The listing builds one solid part. Answer for the finished solid, in the listing's coordinates (mm). Face numbers are marked on the shaded views. A direction names the side the tool comes from. Coordinates: 2 decimals unless noted, no trailing zeros. Loops run counter-clockwise (first coordinate to the right, second up) from the corner with the lowest first, then second, coordinate; pieces in that order, holes last. Notation, with made-up numbers: M -37.75,-37 L -27.75,-37 A24 cw -27.75,-9 Z; hole C -15,-24.75 d8. An arc over 180 degrees is marked long. Answer as a JSON object with one key per item and string values. Group by question number.
1. Straight lines are drawn through the part: L1, parallel to Z at x = 91, y = 9; L2, parallel to X at y = 14.5, z = 6; L3, parallel to Y at x = 291.5, z = -6. For each, find the intervals that lie inside material, in ascending order.
2. A cutting plane is placed at B-B on x = 130.5. Give the vertices of the cut face in (y, z).
3. For the marked faces 1, 2 and 3, determine the directions among +Z, -Z, +X, -X, +Y, -Y from which every point of the face is accessible in a straight line to the end or side of a thin tool.
4. Given pin 1 (1.3 mm diameter, centred on x = -60.5, y = 15.5, fed in from +Z); pin 2 (3 mm diameter, centred on x = -117, z = -2.5, fed in from +Y); pin 3 (3 mm diameter, centred on x = -58.5, z = -2, fed in from +Y); pin 4 (6 mm diameter, centred on y = 0.5, z = 4.5, fed in from +X), each flat-ended and moving along its own axis, determine where each tip first touches the part or whether it passes through.
5. A cutting plane is placed at A-A on x = 53. Give the vertices of the cut face in (y, z), and give its area (3 significant figures).
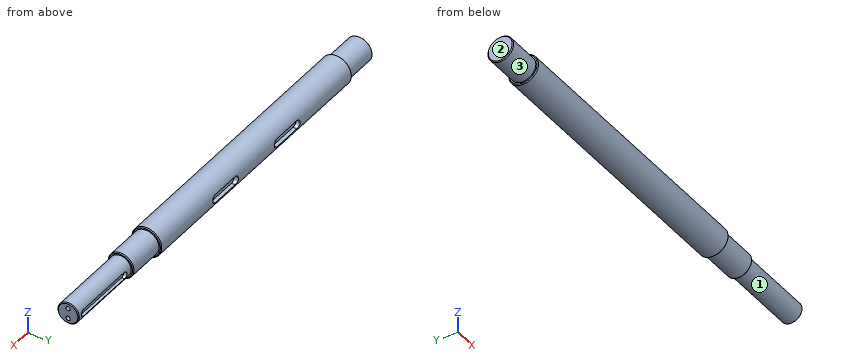
from build123d import *

# Parameters (mm, degrees)
CUT_EXTRUDE_1_DEPTH    = 5
CUT_EXTRUDE_2_DEPTH    = 4
CHAMFER_1_SIZE         = 1
HOLE_WIZARD_M6_1_D     = 5
HOLE_WIZARD_M6_1_DEPTH = 20
HOLE_WIZARD_M6_1_TIP   = 1.502151548


with BuildPart() as part:
    # 草图1 → 旋转1 (revolve)
    with BuildSketch(Plane.XY, mode=Mode.PRIVATE) as revolve_1_sk:
        Polygon((167, 17.5), (0, 17.5), (-167, 17.5), (-167, 15), (-207, 15), (-207, 0), (304, 0), (304, 12.5), (212, 12.5), (212, 15), (167, 15), align=None)
    revolve(revolve_1_sk.sketch.rotate(Axis((0, 0, 0), (-1, 0, 0)), 90), axis=Axis((0, 0, 0), (-1, 0, 0)))

    # 草图2 → 切除-拉伸1 (cut)
    with BuildSketch(Plane(origin=(0, 17.5, 0), x_dir=(1, 0, 0), z_dir=(0, 1, 0))):
        with BuildLine():
            Line((36.5, 5), (71.5, 5))
            ThreePointArc((71.5, 5), (76.5, 0), (71.5, -5))
            Line((71.5, -5), (36.5, -5))
            ThreePointArc((36.5, -5), (31.5, 0), (36.5, 5))
        make_face()
        with BuildLine():
            Line((-36.5, 5), (-71.5, 5))
            ThreePointArc((-71.5, 5), (-76.5, 0), (-71.5, -5))
            Line((-71.5, -5), (-36.5, -5))
            ThreePointArc((-36.5, -5), (-31.5, 0), (-36.5, 5))
        make_face()
    extrude(amount=-CUT_EXTRUDE_1_DEPTH, mode=Mode.SUBTRACT)

    # 草图3 → 切除-拉伸2 (cut)
    with BuildSketch(Plane(origin=(0, 12.5, 0), x_dir=(1, 0, 0), z_dir=(0, 1, 0))):
        with BuildLine():
            Line((223, 4), (295, 4))
            ThreePointArc((295, 4), (299, 0), (295, -4))
            Line((295, -4), (223, -4))
            ThreePointArc((223, -4), (219, 0), (223, 4))
        make_face()
    extrude(amount=-CUT_EXTRUDE_2_DEPTH, mode=Mode.SUBTRACT)

    # 倒角1
    chamfer_1_edges = [part.edges().sort_by_distance(p)[0] for p in [
        (-207, 0, 15),
        (-167, 0, 17.5),
        (167, 0, 17.5),
        (212, 0, 15),
        (304, 0, 12.5),
    ]]
    chamfer(chamfer_1_edges, length=CHAMFER_1_SIZE)

    # M6 螺纹孔1
    with Locations(Plane(origin=(304, 0, 0), x_dir=(0, 0, -1), z_dir=(1, 0, 0))):
        with Locations((6, 0), (-6, 0)):
            Hole(HOLE_WIZARD_M6_1_D / 2, depth=HOLE_WIZARD_M6_1_DEPTH)
            with Locations((0, 0, -(HOLE_WIZARD_M6_1_DEPTH + HOLE_WIZARD_M6_1_TIP / 2))):  # 118° drill point
                Cone(0, HOLE_WIZARD_M6_1_D / 2, HOLE_WIZARD_M6_1_TIP, mode=Mode.SUBTRACT)


solid = part.part
From the geometry:
{
 "1": {"L1": "z = -15.01 to 15.01", "L2": "x = -167 to 167", "L3": "y = -10.97 to -2.5, 2.5 to 10.97"},
 "2": {"outline": "C 0,0 d35"},
 "3": {"face 1": "+X", "face 2": "+Z, -Z, -X, +Y, -Y", "face 3": "-X"},
 "4": {"pin 1": "stops at z = 9.26", "pin 2": "stops at y = 17.47", "pin 3": "stops at y = 12.5", "pin 4": "stops at x = 304"},
 "5": {"outline": "M 12.5,-5 L 12.5,5 L 16.77,5 A17.5 ccw long 16.77,-5 Z", "area": "915 mm²"}
}
